```python
from build123d import *

# Parameters (mm, degrees)
SKETCH1_W                      = 130
SKETCH1_H                      = 130
BOSS_EXTRUDE1_DEPTH            = 8
SKETCH2_R                      = 50
BOSS_EXTRUDE2_DEPTH            = 100
F_14_0_14_DIAMETER_HOLE1_D     = 14
F_14_0_14_DIAMETER_HOLE1_DEPTH = 22
F_14_0_14_DIAMETER_HOLE1_TIP   = 4.206024333


with BuildPart() as part:
    # Sketch1 → Boss-Extrude1 (new body)
    with BuildSketch(Plane(origin=(0, 0, 0), x_dir=(1, 0, 0), z_dir=(0, 1, 0))):
        Rectangle(SKETCH1_W, SKETCH1_H)
    extrude(amount=BOSS_EXTRUDE1_DEPTH)

    # Sketch2 → Boss-Extrude2 (add)
    with BuildSketch(Plane(origin=(0, 8, 0), x_dir=(1, 0, 0), z_dir=(0, 1, 0))):
        with Locations(Location((0, 0, 0), (0, 0, 270))):
            Circle(SKETCH2_R)
    extrude(amount=BOSS_EXTRUDE2_DEPTH)

    # Ø14.0 (14) Diameter Hole1
    with Locations(Plane(origin=(0, 8, 0), x_dir=(1, 0, 0), z_dir=(0, 1, 0))):
        with Locations((-50, 50), (50, 50), (50, -50), (-50, -50)):
            Hole(F_14_0_14_DIAMETER_HOLE1_D / 2, depth=F_14_0_14_DIAMETER_HOLE1_DEPTH)
            with Locations((0, 0, -(F_14_0_14_DIAMETER_HOLE1_DEPTH + F_14_0_14_DIAMETER_HOLE1_TIP / 2))):  # 118° drill point
                Cone(0, F_14_0_14_DIAMETER_HOLE1_D / 2, F_14_0_14_DIAMETER_HOLE1_TIP, mode=Mode.SUBTRACT)


solid = part.part
```
Could you check a few things on this model? Use its own coordinates, in mm. A direction names the side the tool comes from. Round coordinates to 2 decimals unless told otherwise and drop trailing zeros. Order: outer loops, then holes, each group sorted by start corner. A loop starts at its lowest first (then second) coordinate and runs counter-clockwise, first axis right, second up. Notation, with made-up numbers: M 13.25,-8 L 53.25,-8 A12 ccw 53.25,9 Z; hole C -37,23.5 d5. An arc over 180 degrees is marked long. One line per question, with ' | ' between items. Start each with the question number.
(1) For P1, Ø1, axis at y = 42, z = -46, coming from the +X side; P2, Ø5, axis at y = 44.5, z = 27.5, coming from the +X side; P3, Ø12, axis at x = 30, y = 20.5, coming from the -Z side, each with a flat end and sliding along its axis, tell me the tip position at first contact or that it passes through.
(2) Thinking about a two-plate mould opening in X: for faces 3 (the face through (-65, 4, 1)), 4 (the face through (43.323, 3.944, -52.103)), 5 (the face through (-1, 4, 65)), which applies, +X half, -X half, draft (parallel to the pull), parting line (faces both ways), or undercut?
(3) Suppose I cut it at B-B on x = 0. List the corners of the cut face in (y, z) for me.
(4) Suppose I cut it at C-C on z = 29. List the corners of the cut face in (x, y) for me, then the cut area to 3 significant figures.
(5) Suppose I cut it at D-D on y = 50.5. List the corners of the cut face in (x, z) for me.
(6) Suppose I cut it at A-A on z = 47.5. List the corners of the cut face in (x, y) for me.
(7) For faces 1 (the face through (-44, 8, -30)), 2 (the face through (46.237, 3.944, 44.098)), which set-ups out of +Z, -Z, +X, -X, +Y, -Y let a thin tool reach every point of the face, with its end or its side?
(8) Please list where these lines run through material, in increasing order: line 1 along X through (y, z) = (3, 50); line 2 along Y through (x, z) = (-7, -56.5).
Geometry results:
1) P1: x = 20.73 | P2: x = 43.3 | P3: z = -43.86
2) face 3: -X half | face 4: undercut | face 5: draft
3) outline: M 0,-65 L 8,-65 L 8,-50 L 108,-50 L 108,50 L 8,50 L 8,65 L 0,65 Z
4) outline: M -65,0 L 65,0 L 65,8 L 40.73,8 L 40.73,108 L -40.73,108 L -40.73,8 L -65,8 Z | area: 9,190 mm²
5) outline: C 0,0 d100
6) outline: M -65,0 L -56.54,0 L -56.54,8 L -65,8 Z; M -43.46,0 L 43.46,0 L 43.46,8 L 15.61,8 L 15.61,108 L -15.61,108 L -15.61,8 L -43.46,8 Z; M 56.54,0 L 65,0 L 65,8 L 56.54,8 Z
7) face 1: +Y | face 2: +Y, -Y
8) line 1: -65 to -57, -43 to 43, 57 to 65 | line 2: 0 to 8
